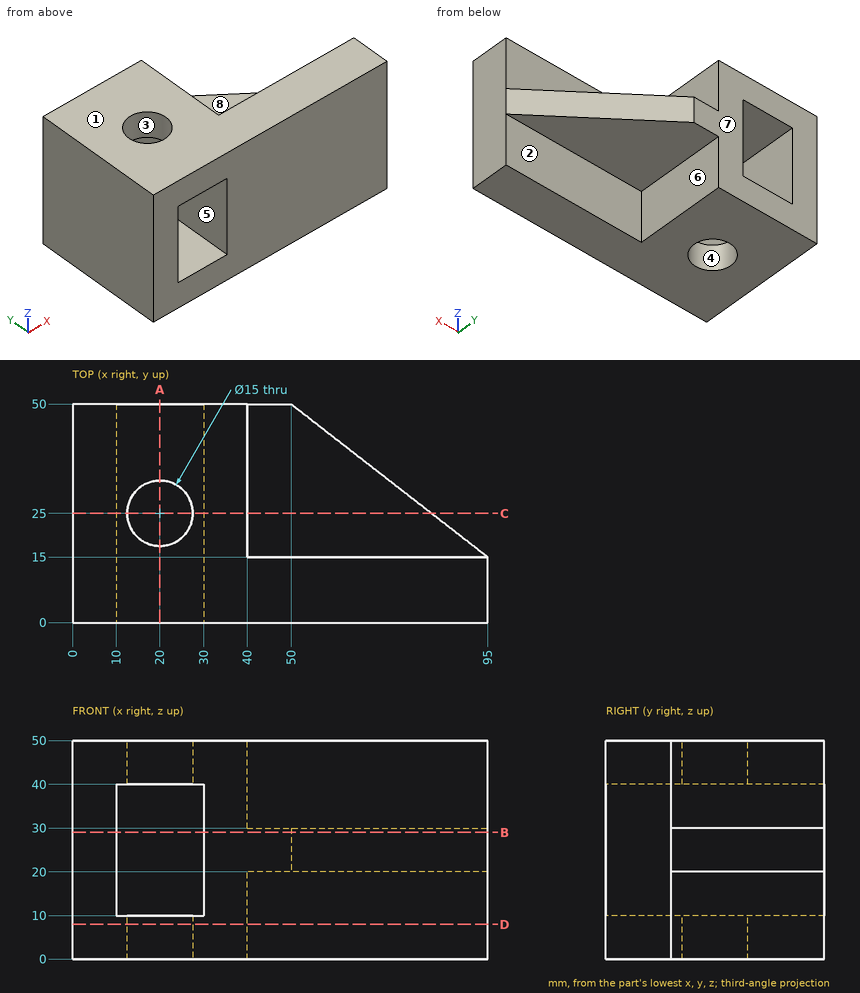
The drawing under review shows one solid part. Ordinate dimensions are in mm from its lowest x, y, z. A direction names the side the tool comes from. Round coordinates to 2 decimals unless told otherwise and drop trailing zeros. Loops run counter-clockwise (first coordinate to the right, second up) from the corner with the lowest first, then second, coordinate; pieces in that order, holes last. Notation, with made-up numbers: (31, 14.25) - (78, 14.25) arc R14 cw to (78, 35.25) - close; hole circle Ø6 at (80.5, -37.75). An arc over 180 degrees is marked (long way). One line per item, written item: value. Start each with the question number.
1) To check wall thickness, follow L1, parallel to Y at x = 20, z = 8; L2, parallel to X at y = 13, z = 25.5; L3, parallel to X at y = 25, z = 3.5. State the ranges of each line that lie inside material, in increasing order. Write a range as from..to.
2) For the marked faces 4, 5, 6, 7 and 8, list the 3-axis set-ups (+Z, -Z, +X, -X, +Y, -Y) from which the entire face can be reached by the end or side of a thin tool; tool diameter is ignored.
3) Consider section D-D on z = 8. Give the boundary of the cut face in (x, y).
4) Consider section C-C on y = 25. Give the boundary of the cut face in (x, z), then the cut area to 3 significant figures.
5) Insertion check: pin 1 Ø5 at (y, z) = (36, 40.5) entering from +X; pin 2 Ø1.5 at (x, y) = (58.5, 44.5) entering from +Z; pin 3 Ø10 at (x, z) = (67.5, 43.5) entering from +Y; pin 4 Ø5 at (x, z) = (63.5, 23) entering from +Y. Each pin has a flat end and moves straight along its axis. Give the tip position at first contact, or say it passes through.
6) Draft analysis for pull direction Y (two halves, no side actions). For the marked faces 1, 2 and 3, state which applies: +Y half, -Y half, draft (parallel to the pull), parting line (faces both ways), or undercut.
7) Consider section B-B on z = 29. Give the boundary of the cut face in (x, y).
8) Consider section A-A on x = 20. Give the boundary of the cut face in (y, z).
Reported:
1. L1: y = 0..17.5, 32.5..50
1. L2: x = 0..10, 30..95
1. L3: x = 0..12.5, 27.5..40
2. face 4: +Z, -Z
2. face 5: +Y, -Y
2. face 6: -Z, +X, +Y
2. face 7: +Z, -Z, +X, -X, +Y
2. face 8: +Z, +X, +Y
3. outline: (0, 0) - (95, 0) - (95, 15) - (40, 15) - (40, 50) - (0, 50) - close; hole circle Ø15 at (20, 25)
4. outline: (0, 0) - (12.5, 0) - (12.5, 10) - (10, 10) - (10, 40) - (12.5, 40) - (12.5, 50) - (0, 50) - close; (27.5, 0) - (40, 0) - (40, 20) - (82.14, 20) - (82.14, 30) - (40, 30) - (40, 50) - (27.5, 50) - (27.5, 40) - (30, 40) - (30, 10) - (27.5, 10) - close
4. area: 1,520 mm^2
5. pin 1: stops at x = 40
5. pin 2: passes through
5. pin 3: stops at y = 15
5. pin 4: stops at y = 41.44
6. face 1: draft
6. face 2: +Y half
6. face 3: undercut
7. outline: (0, 0) - (10, 0) - (10, 50) - (0, 50) - close; (30, 0) - (95, 0) - (95, 15) - (50, 50) - (30, 50) - close
8. outline: (0, 0) - (17.5, 0) - (17.5, 10) - (0, 10) - close; (0, 40) - (17.5, 40) - (17.5, 50) - (0, 50) - close; (32.5, 0) - (50, 0) - (50, 10) - (32.5, 10) - close; (32.5, 40) - (50, 40) - (50, 50) - (32.5, 50) - close
